from build123d import *

# Parameters (mm, degrees)
SKETCH2_R                = 38.5
SKETCH2_R_2              = 29
SKETCH2_R_3              = 1.85
BOSS_EXTRUDE1_DEPTH      = 8
BOSS_EXTRUDE2_DEPTH      = 5
BOSS_EXTRUDE2_DEPTH_BACK = 5
SKETCH4_W                = 22.91440569
SKETCH4_H                = 10
SKETCH4_W_2              = 25.697687416
BOSS_EXTRUDE3_DEPTH      = 8
CUT_EXTRUDE1_REACH       = 122.328
SKETCH5_R                = 5
FILLET1_R                = 7
CUT_EXTRUDE2_REACH       = 122.328
SKETCH6_W                = 76.347887986
SKETCH6_H                = 64.488526755


with BuildPart() as part:
    # Sketch2 → Boss-Extrude1 (new body)
    with BuildSketch(Plane.XY):
        Circle(SKETCH2_R)
        with Locations((0.678631435, 0)):
            Circle(SKETCH2_R_2, mode=Mode.SUBTRACT)
        with Locations((0, 34.5)):
            Circle(SKETCH2_R_3, mode=Mode.SUBTRACT)
        with Locations((24.395183951, 24.395183951)):
            Circle(SKETCH2_R_3, mode=Mode.SUBTRACT)
        with Locations((24.395183951, -24.395183951)):
            Circle(SKETCH2_R_3, mode=Mode.SUBTRACT)
        with Locations((0, -34.5)):
            Circle(SKETCH2_R_3, mode=Mode.SUBTRACT)
        with Locations((-24.395183951, -24.395183951)):
            Circle(SKETCH2_R_3, mode=Mode.SUBTRACT)
        with Locations((-24.395183951, 24.395183951)):
            Circle(SKETCH2_R_3, mode=Mode.SUBTRACT)
    extrude(amount=BOSS_EXTRUDE1_DEPTH)

    # Sketch3 → Boss-Extrude2 (add, two sides: drawn at the far end of the back side and taken through both)
    with BuildSketch(Plane(origin=(0, 0, 0), x_dir=(1, 0, 0), z_dir=(0, 1, 0)).offset(-BOSS_EXTRUDE2_DEPTH_BACK)):
        Polygon((-28.321368565, 0), (-38.5, 0), (-58.321368565, 0), (-58.321368565, 67.772616809), (-58.321368565, 95), (59.678631435, 95), (59.678631435, 67.772616809), (59.678631435, 0), (38.5, 0), (29.678631435, 0), (29.678631435, 60), (-28.321368565, 60), align=None)
    extrude(amount=BOSS_EXTRUDE2_DEPTH + BOSS_EXTRUDE2_DEPTH_BACK)

    # Sketch4 → Boss-Extrude3 (add)
    with BuildSketch(Plane.XY):
        with Locations((-46.86416572, 0)):
            Rectangle(SKETCH4_W, SKETCH4_H)
        with Locations((46.829787727, 0)):
            Rectangle(SKETCH4_W_2, SKETCH4_H)
    extrude(amount=BOSS_EXTRUDE3_DEPTH)

    # Sketch5 → Cut-Extrude1 (cut, up to next)
    with BuildSketch(Plane(origin=(0, 5, 0), x_dir=(1, 0, 0), z_dir=(0, 1, 0)), mode=Mode.PRIVATE) as cut_extrude1_sk1:
        with Locations(Location((-46.321368565, 83, 0), (0, 0, 270))):
            Circle(SKETCH5_R)
    cut_extrude1_tool1 = extrude(cut_extrude1_sk1.sketch, amount=-CUT_EXTRUDE1_REACH, mode=Mode.PRIVATE) & part.part
    # Sketch5 → Cut-Extrude1 (cut, up to next)
    with BuildSketch(Plane(origin=(0, 5, 0), x_dir=(1, 0, 0), z_dir=(0, 1, 0)), mode=Mode.PRIVATE) as cut_extrude1_sk2:
        with Locations(Location((-46.321368565, 4, 0), (0, 0, 270))):
            Circle(SKETCH5_R)
    cut_extrude1_tool2 = extrude(cut_extrude1_sk2.sketch, amount=-CUT_EXTRUDE1_REACH, mode=Mode.PRIVATE) & part.part
    # Sketch5 → Cut-Extrude1 (cut, up to next)
    with BuildSketch(Plane(origin=(0, 5, 0), x_dir=(1, 0, 0), z_dir=(0, 1, 0)), mode=Mode.PRIVATE) as cut_extrude1_sk3:
        with Locations(Location((47.678631435, 83, 0), (0, 0, 270))):
            Circle(SKETCH5_R)
    cut_extrude1_tool3 = extrude(cut_extrude1_sk3.sketch, amount=-CUT_EXTRUDE1_REACH, mode=Mode.PRIVATE) & part.part
    # Sketch5 → Cut-Extrude1 (cut, up to next)
    with BuildSketch(Plane(origin=(0, 5, 0), x_dir=(1, 0, 0), z_dir=(0, 1, 0)), mode=Mode.PRIVATE) as cut_extrude1_sk4:
        with Locations(Location((47.678631435, 4, 0), (0, 0, 270))):
            Circle(SKETCH5_R)
    cut_extrude1_tool4 = extrude(cut_extrude1_sk4.sketch, amount=-CUT_EXTRUDE1_REACH, mode=Mode.PRIVATE) & part.part
    add(cut_extrude1_tool1.solids().sort_by_distance((-46.321369, 5, -83))[0], mode=Mode.SUBTRACT)
    add(cut_extrude1_tool2.solids().sort_by_distance((-46.321369, 5, -4))[0], mode=Mode.SUBTRACT)
    add(cut_extrude1_tool3.solids().sort_by_distance((47.678631, 5, -83))[0], mode=Mode.SUBTRACT)
    add(cut_extrude1_tool4.solids().sort_by_distance((47.678631, 5, -4))[0], mode=Mode.SUBTRACT)

    # Fillet1
    fillet1_edges = [part.edges().sort_by_distance(p)[0] for p in [
        (-28.321368565, 0, -60),
        (-58.321368565, 0, -95),
        (59.678631435, 0, -95),
        (29.678631435, 0, -60),
        (-58.321368565, 0, 8),
        (59.678631435, 0, 8),
    ]]
    fillet(fillet1_edges, radius=FILLET1_R)

    # Sketch6 → Cut-Extrude2 (cut, up to next)
    with BuildSketch(Plane(origin=(0, 5, 0), x_dir=(1, 0, 0), z_dir=(0, 1, 0)), mode=Mode.PRIVATE) as cut_extrude2_sk1:
        with Locations((0, 32.244263378)):
            Rectangle(SKETCH6_W, SKETCH6_H)
    cut_extrude2_tool1 = extrude(cut_extrude2_sk1.sketch, amount=-CUT_EXTRUDE2_REACH, mode=Mode.PRIVATE) & part.part
    add(cut_extrude2_tool1.solids().sort_by_distance((0, 5, -32.244263))[0], mode=Mode.SUBTRACT)


solid = part.part
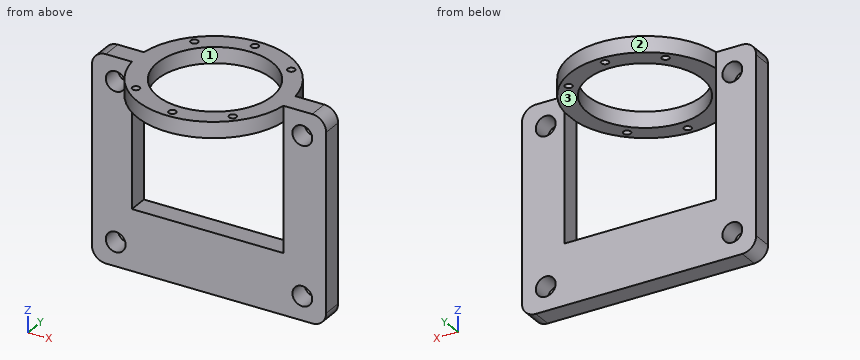
Build history of the part. All positions in model axes, mm. Face numbers are marked on the shaded views. Round coordinates to 2 decimals unless told otherwise and drop trailing zeros. Loops run counter-clockwise (first coordinate to the right, second up) from the corner with the lowest first, then second, coordinate; pieces in that order, holes last. Notation, with made-up numbers: (-10.75, 64.5) -> (40.25, 64.5) arc R21 cw to (40.25, 96.5) -> close; hole circle Ø2 at (84, 60). An arc over 180 degrees is marked (long way). Answer in a Markdown table with one row per item.
Item 1: Mould opens along Y. For the marked faces 1, 2 and 3 say: +Y half, -Y half, draft (parallel to the pull), parting line (faces both ways), or undercut.
Answers below:
| item | result |
|---|---|
| face 1 | undercut |
| face 2 | +Y half |
| face 3 | draft |
Item 2: Saw through at D-D (y = 16). Write the cut outline in (x, z).
Answers below:
| item | result |
|---|---|
| outline | (-35.02, 0) -> (-23.51, 0) -> (-23.51, 8) -> (-35.02, 8) -> close; (24.87, 0) -> (35.02, 0) -> (35.02, 8) -> (24.87, 8) -> close |
Item 3: Drill centre lines: L1, parallel to X at y = 4, z = -3.5; L2, parallel to Y at x = 0, z = 2.25; L3, parallel to Z at x = 45, y = 4. Where is each one in solid material? Low to high. Write a range as [from, to].
Answers below:
| item | result |
|---|---|
| L1 | x = [-58.32, -51.3], [-41.35, -38.17], [38.17, 42.7], [52.65, 59.68] |
| L2 | y = [-38.5, -36.35], [-32.65, -28.99], [28.99, 32.65], [36.35, 38.5] |
| L3 | z = [-95, -87.22], [-78.78, -8.22], [0.22, 8] |
Item 4: Saw through at B-B (z = -83). Write the cut outline in (x, y), and give its area (3 significant figures).
Answers below:
| item | result |
|---|---|
| outline | (-58.32, -5) -> (-51.32, -5) -> (-51.32, 5) -> (-58.32, 5) -> close; (-41.32, -5) -> (42.68, -5) -> (42.68, 5) -> (-41.32, 5) -> close; (52.68, -5) -> (59.68, -5) -> (59.68, 5) -> (52.68, 5) -> close |
| area | 980 mm² |
Item 5: Saw through at A-A (z = -52.5). Write the cut outline in (x, y).
Answers below:
| item | result |
|---|---|
| outline | (-58.32, -5) -> (-38.17, -5) -> (-38.17, 5) -> (-58.32, 5) -> close; (38.17, -5) -> (59.68, -5) -> (59.68, 5) -> (38.17, 5) -> close |
Item 6: Saw through at C-C (x = -19.5). Write the cut outline in (y, z), and give its area (3 significant figures).
Answers below:
| item | result |
|---|---|
| outline | (-33.2, 0) -> (-20.83, 0) -> (-20.83, 8) -> (-33.2, 8) -> close; (-5, -95) -> (5, -95) -> (5, -64.49) -> (-5, -64.49) -> close; (20.83, 0) -> (33.2, 0) -> (33.2, 8) -> (20.83, 8) -> close |
| area | 503 mm² |
Item 7: Pin check, flat tips, straight feed: pin 1 (16 mm diameter, centred on x = -46.32, z = -4, fed in from -Y); pin 2 (3 mm diameter, centred on x = 24.4, y = 24.4, fed in from +Z); pin 3 (11.5 mm diameter, centred on x = -46.32, z = -83, fed in from +Y); pin 4 (10 mm diameter, centred on x = -38, y = -15, fed in from -Z). Stop position of each tip, or through.
Answers below:
| item | result |
|---|---|
| pin 1 | stops at y = -5 |
| pin 2 | passes through |
| pin 3 | stops at y = 5 |
| pin 4 | stops at z = 0 |
